Geometry: see drawing. Coordinates: mm, zero at the bounding-box minimum. A direction names the side the tool comes from. Coordinates: 2 decimals unless noted, no trailing zeros. Write each loop counter-clockwise with the first axis right and the second up, starting at its lowest first coordinate (ties: lowest second). Pieces come first, ordered by that corner, then holes. Notation, with made-up numbers: (49, 48.25) - (64, 48.25) arc R19 ccw to (64, 59.25) - close; hole circle Ø9 at (-29.5, 62). An arc over 180 degrees is marked (long way). One line per question, with ' | ' between items. Start each with the question number.
1) First-contact query: P1, Ø9, axis at x = 90, y = 44, coming from the +Z side; P2, Ø24, axis at x = 68.5, y = 23.5, coming from the -Z side; P3, Ø4, axis at x = 10, y = 6, coming from the -Z side. Flat tips, straight axial feed; report the tip coordinate or a pass-through.
2) Section query C-C on z = 13.75. Return loops of the section in (x, y), and give its area (3 significant figures).
3) Section query B-B on y = 44. Return loops of the section in (x, z).
4) Line query: line 1 (Y direction, x = 10, z = 10); line 2 (X direction, y = 41, z = 7.75); line 3 (Z direction, x = 29, y = 16.5). Output: solid intervals per line, ascending.
5) Section query D-D on x = 78.5. Return loops of the section in (y, z), and give its area (3 significant figures).
6) Reachability of the marked faces 1 and 2 from +Z, -Z, +X, -X, +Y, -Y: full face, straight path, thin tool, end or side. Return the list, or none.
7) Section query A-A on x = 90. Return loops of the section in (y, z), and give its area (3 significant figures).
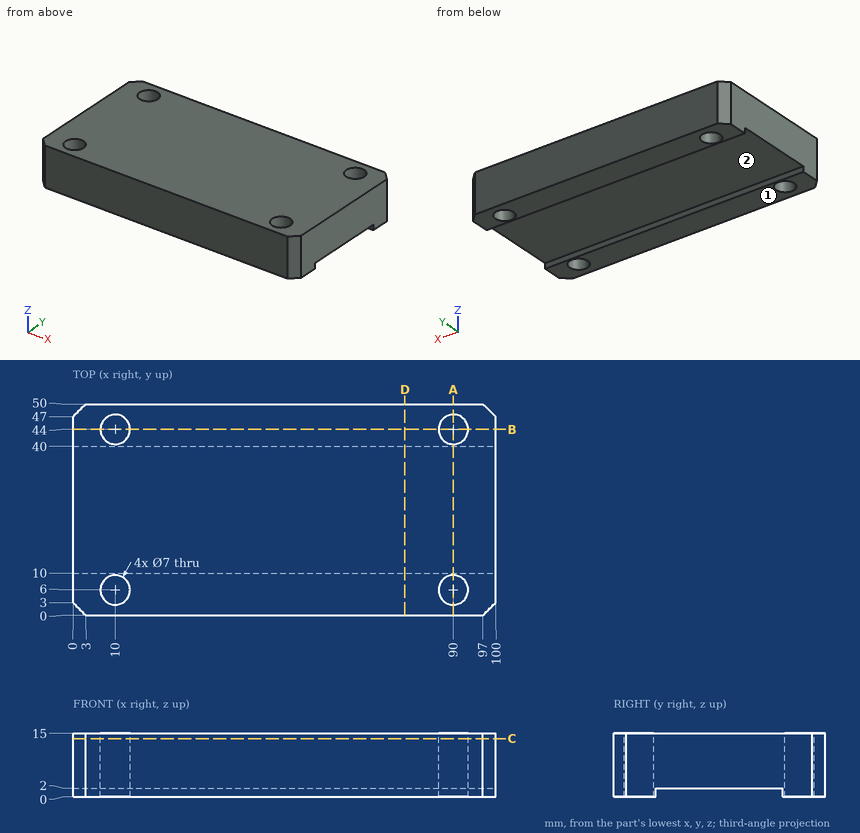
Answer key:
1) P1: z = 15 | P2: z = 2 | P3: through
2) outline: (0, 3) - (3, 0) - (97, 0) - (100, 3) - (100, 47) - (97, 50) - (3, 50) - (0, 47) - close; hole circle Ø7 at (10, 6); hole circle Ø7 at (10, 44); hole circle Ø7 at (90, 6); hole circle Ø7 at (90, 44) | area: 4,830 mm²
3) outline: (0, 0) - (6.5, 0) - (6.5, 15) - (0, 15) - close; (13.5, 0) - (86.5, 0) - (86.5, 15) - (13.5, 15) - close; (93.5, 0) - (100, 0) - (100, 15) - (93.5, 15) - close
4) line 1: 0 to 2.5, 9.5 to 40.5, 47.5 to 50 | line 2: 0 to 8.2, 11.8 to 88.2, 91.8 to 100 | line 3: 2 to 15
5) outline: (0, 0) - (10, 0) - (10, 2) - (40, 2) - (40, 0) - (50, 0) - (50, 15) - (0, 15) - close | area: 690 mm²
6) face 1: -Z, +X, -X, +Y, -Y | face 2: -Z, +X, -X
7) outline: (0, 0) - (2.5, 0) - (2.5, 15) - (0, 15) - close; (9.5, 0) - (10, 0) - (10, 2) - (40, 2) - (40, 0) - (40.5, 0) - (40.5, 15) - (9.5, 15) - close; (47.5, 0) - (50, 0) - (50, 15) - (47.5, 15) - close | area: 480 mm²
